Answer from the drawing. Dimensions are ordinates in mm from the lowest x, y and z of the part. Coordinates: 2 decimals unless noted, no trailing zeros. Order: outer loops, then holes, each group sorted by start corner. A loop starts at its lowest first (then second) coordinate and runs counter-clockwise, first axis right, second up. Notation, with made-up numbers: M 27.5,-0.5 L 31.5,-0.5 A13 cw 31.5,19.5 Z; hole C 31.25,61.25 d6. An arc over 180 degrees is marked long. Write each question's results on one line, items separated by ' | '.
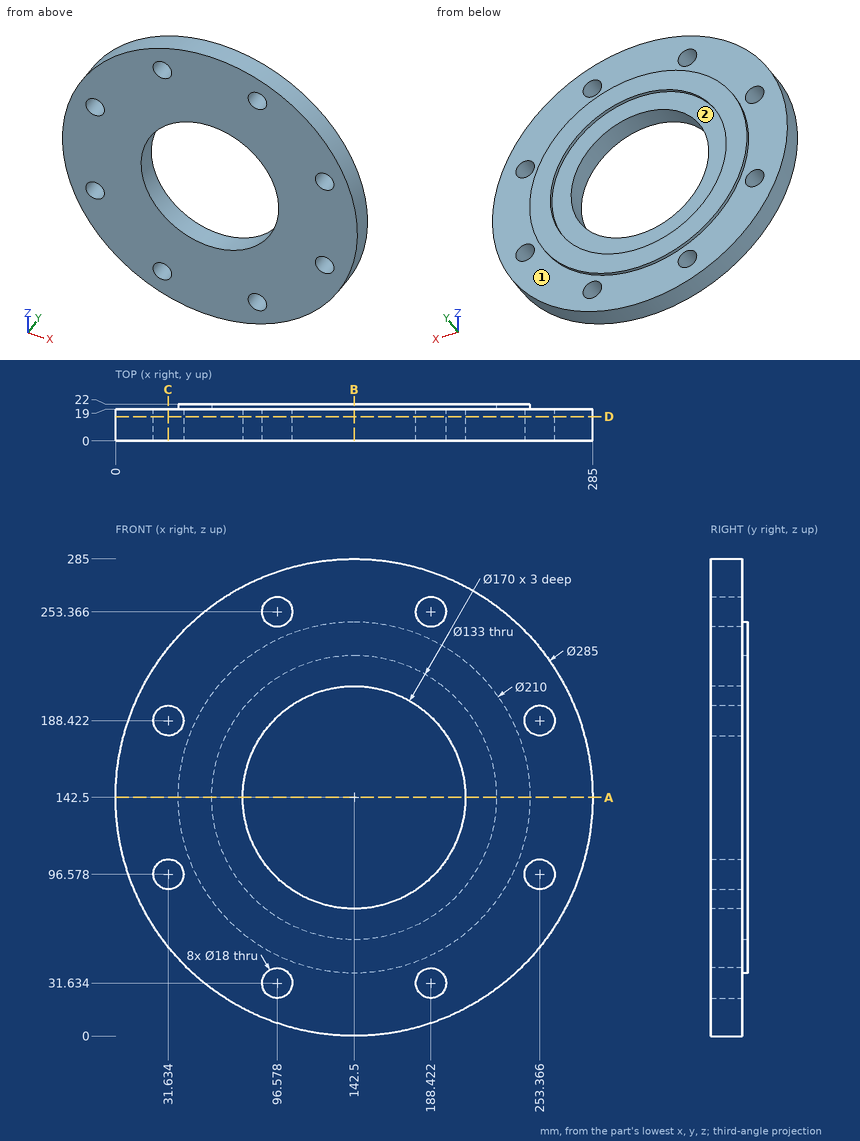
(1) Given pin 1 (20.5 mm diameter, centred on x = 96.58, z = 31.63, fed in from -Y); pin 2 (5 mm diameter, centred on y = 12, z = 95, fed in from +X); pin 3 (5 mm diameter, centred on x = 164, y = 8.5, fed in from -Z); pin 4 (16 mm diameter, centred on x = 253.37, z = 96.58, fed in from +Y), each flat-ended and moving along its own axis, determine where each tip first touches the part or whether it passes through.
Conclusion:
pin 1: y = 0 | pin 2: x = 277.71 | pin 3: z = 1.27 | pin 4: through
(2) The part is cut by section D-D, the plane y = 14.5. Count the separate pieces of the cut face and the enclosed holes in it, then the cut area to 3 significant figures.
Conclusion:
separate pieces: 1 | enclosed holes: 9 | area: 47,900 mm²
(3) The part is cut by section A-A, the plane z = 142.5. Write down the section's boundary in (x, y), then the cut area to 3 significant figures.
Conclusion:
outline: M 0,0 L 76,0 L 76,19 L 57.5,19 L 57.5,22 L 37.5,22 L 37.5,19 L 0,19 Z; M 209,0 L 285,0 L 285,19 L 247.5,19 L 247.5,22 L 227.5,22 L 227.5,19 L 209,19 Z | area: 3,010 mm²
(4) The mould has two halves that part along X. Classify the marked faces 1 and 2: pulls with the +X half, pulls with the -X half, needs draft (parallel to the pull), parting line crosses it, or undercut.
Conclusion:
face 1: needs draft | face 2: undercut
(5) The part is cut by section B-B, the plane x = 142.5. Write down the section's boundary in (y, z), then the cut area to 3 significant figures.
Conclusion:
outline: M 0,0 L 19,0 L 19,37.5 L 22,37.5 L 22,57.5 L 19,57.5 L 19,76 L 0,76 Z; M 0,209 L 19,209 L 19,227.5 L 22,227.5 L 22,247.5 L 19,247.5 L 19,285 L 0,285 Z | area: 3,010 mm²
(6) The part is cut by section C-C, the plane x = 31.5. Write down the section's boundary in (y, z).
Conclusion:
outline: M 0,53.14 L 19,53.14 L 19,87.58 L 0,87.58 Z; M 0,105.58 L 19,105.58 L 19,179.42 L 0,179.42 Z; M 0,197.42 L 19,197.42 L 19,231.86 L 0,231.86 Z
(7) Straight lines are drawn through the part: line 1 (Z direction, x = 140, y = 15); line 2 (X direction, y = 9.75, z = 101) (1 decimal); line 3 (X direction, y = 15.75, z = 94) (1 decimal). For each, find the intervals that lie inside material, in ascending order.
Conclusion:
line 1: 0.02 to 76.05, 208.95 to 284.98 | line 2: 6.2 to 23.8, 39.5 to 90.5, 194.5 to 245.5, 261.2 to 278.8 | line 3: 8.5 to 23, 40.3 to 97, 188 to 244.7, 262 to 276.5
